Source: CAD feature listing. Evaluate the final solid. Frame: model axes, mm. A direction names the side the tool comes from. Give positions to 0.01 mm unless a question says otherwise; leave off trailing zeros. Write each loop counter-clockwise with the first axis right and the second up, starting at its lowest first coordinate (ties: lowest second). Pieces come first, ordered by that corner, then holes. Notation, with made-up numbers: M 70,-1 L 109,-1 A25 ccw 109,35 Z; hole C 75,-35 d10. An arc over 180 degrees is marked long. Return JSON: item names as keys, results as strings.
```python
from build123d import *

# Parameters (mm, degrees)
SKETCH1_W           = 68
SKETCH1_H           = 225
BOSS_EXTRUDE1_DEPTH = 5
SKETCH3_R           = 7.6
CUT_EXTRUDE1_DEPTH  = 8
FILLET1_R           = 8
CUT_EXTRUDE2_DEPTH  = 118.631840928
FILLET2_R           = 10
CUT_EXTRUDE3_DEPTH  = 8
FILLET3_R           = 10
CUT_EXTRUDE4_DEPTH  = 118.631840928
FILLET4_R           = 5
FILLET5_R           = 50


with BuildPart() as part:
    # Sketch1 → Boss-Extrude1 (new body)
    with BuildSketch(Plane.XY):
        Rectangle(SKETCH1_W, SKETCH1_H)
    extrude(amount=BOSS_EXTRUDE1_DEPTH)

    # Sketch3 → Cut-Extrude1 (cut)
    with BuildSketch(Plane.XY.offset(5)):
        with Locations((22.5, -102.5)):
            Circle(SKETCH3_R)
        with Locations((10.929823026, -88.711200024)):
            Circle(SKETCH3_R)
        with Locations((-0.640353949, -74.922400048)):
            Circle(SKETCH3_R)
        with Locations((-12.210530923, -61.133600072)):
            Circle(SKETCH3_R)
        with Locations((-23.780707897, -47.344800095)):
            Circle(SKETCH3_R)
    extrude(amount=-CUT_EXTRUDE1_DEPTH, mode=Mode.SUBTRACT)

    # Fillet1
    fillet1_edges = [part.edges().sort_by_distance(p)[0] for p in [
        (34, -112.5, 2.5),
    ]]
    fillet(fillet1_edges, radius=FILLET1_R)

    # Sketch5 → Cut-Extrude2 (cut, through all)
    with BuildSketch(Plane.XY.offset(5)):
        Polygon((14.573405195, -112.5), (-34, -54.612469854), (-34, -112.5), align=None)
    extrude(amount=-CUT_EXTRUDE2_DEPTH, mode=Mode.SUBTRACT)

    # Fillet2
    fillet2_edges = [part.edges().sort_by_distance(p)[0] for p in [
        (14.573405195, -112.5, 2.5),
    ]]
    fillet(fillet2_edges, radius=FILLET2_R)

    # Sketch6 → Cut-Extrude3 (cut)
    with BuildSketch(Plane.XY.offset(5)):
        with BuildLine():
            Line((-11, 112.5), (-11, 98.643593539))
            ThreePointArc((-11, 98.643593539), (0, 92.57179677), (11, 98.643593539))
            Line((11, 98.643593539), (11, 112.5))
            ThreePointArc((11, 112.5), (0, 118.57179677), (-11, 112.5))
        make_face()
    extrude(amount=-CUT_EXTRUDE3_DEPTH, mode=Mode.SUBTRACT)

    # Fillet3
    fillet3_edges = [part.edges().sort_by_distance(p)[0] for p in [
        (-34, -54.612469854, 2.5),
    ]]
    fillet(fillet3_edges, radius=FILLET3_R)

    # Sketch7 → Cut-Extrude4 (cut, through all)
    with BuildSketch(Plane.XY.offset(5)):
        Polygon((-20, 112.5), (-34, 52.5), (-34, 112.5), align=None)
        Polygon((34, 112.5), (20, 112.5), (34, 52.5), align=None)
    extrude(amount=-CUT_EXTRUDE4_DEPTH, mode=Mode.SUBTRACT)

    # Fillet4
    fillet4_edges = [part.edges().sort_by_distance(p)[0] for p in [
        (20, 112.5, 2.5),
        (-20, 112.5, 2.5),
    ]]
    fillet(fillet4_edges, radius=FILLET4_R)

    # Fillet5
    fillet5_edges = [part.edges().sort_by_distance(p)[0] for p in [
        (34, 52.5, 2.5),
        (-34, 52.5, 2.5),
    ]]
    fillet(fillet5_edges, radius=FILLET5_R)


solid = part.part
```
1) Line query: line 1 (Y direction, x = -18, z = 3.9); line 2 (Y direction, x = 4.5, z = 0.6); line 3 (Y direction, x = -1, z = 4). Output: solid intervals per line, ascending. Write a range as [from, to].
Numbers:
{"line 1": "y = [-73.68, -66.06], [-56.21, -52.28], [-42.41, 112.1]", "line 2": "y = [-100.49, -92.76], [-84.66, -80.52], [-69.32, 93.38]", "line 3": "y = [-93.94, -82.51], [-67.33, 92.61]"}
2) Cut plane B-B, the plane x = -24.5. Return the cut outline in (y, z).
Numbers:
{"outline": "M -65.93,0 L -54.91,0 L -54.91,5 L -65.93,5 Z; M -39.78,0 L 93.21,0 L 93.21,5 L -39.78,5 Z"}
3) Cut plane D-D, the plane y = 80. Return the cut outline in (x, z).
Numbers:
{"outline": "M -27.58,0 L 27.58,0 L 27.58,5 L -27.58,5 Z"}
4) Cut plane C-C, the plane z = 1.1. Return the cut outline in (x, y).
Numbers:
{"outline": "M -34,-50.97 A10 ccw -31.66,-57.4 L 11.58,-108.93 A10 ccw 19.24,-112.5 L 26,-112.5 A8 ccw 34,-104.5 L 34,46.74 A50 ccw 32.69,58.11 L 20.9,108.64 A5 ccw 16.03,112.5 L 11,112.5 L 11,98.64 A13 cw -11,98.64 L -11,112.5 L -16.03,112.5 A5 ccw -20.9,108.64 L -32.69,58.11 A50 ccw -34,46.74 Z; hole C -23.78,-47.34 d15.2; hole C -12.21,-61.13 d15.2; hole C -0.64,-74.92 d15.2; hole C 10.93,-88.71 d15.2; hole C 22.5,-102.5 d15.2"}
5) Draft query along Y for faces 3 (the face through (13, 112.5, 2)), 4 (the face through (11, 105, 3)), 5 (the face through (-13.858, -68.553, 2.535)). Return one class per face: released by +Y, released by -Y, zero draft, split by the parting line, or undercut.
Numbers:
{"face 3": "released by +Y", "face 4": "zero draft", "face 5": "undercut"}
6) Set-up query: faces 1 (the face through (-11, 106, 3)), 2 (the face through (-33.663, 52.542, 2.465)). Return all of +Z, -Z, +X, -X, +Y, -Y with unobstructed straight access to the full face (end or side cutting, diameter ignored); none if empty.
Numbers:
{"face 1": "+Z, -Z, +Y", "face 2": "+Z, -Z, -X, +Y"}
7) Contact query for flat-ended pins moving along their axis: pin 1 Ø12 at (x, y) = (22.5, -102.5) entering from +Z; pin 2 Ø2.5 at (y, z) = (104, 3) entering from -X (3 decimals); pin 3 Ø1.5 at (y, z) = (107, 2.5) entering from +X; pin 4 Ø1.5 at (y, z) = (75.5, 3.5) entering from -X. Output: stop coordinate, or through.
Numbers:
{"pin 1": "passes through", "pin 2": "stops at x = -22.275", "pin 3": "stops at x = 21.46", "pin 4": "stops at x = -28.81"}
8) Cut plane A-A, the plane y = -86.5. Return the cut outline in (x, z), then the cut area to 3 significant figures.
Numbers:
{"outline": "M -7.24,0 L 3.66,0 L 3.66,5 L -7.24,5 Z; M 18.2,0 L 34,0 L 34,5 L 18.2,5 Z", "area": "134 mm²"}
